from build123d import *

# Parameters (mm, degrees)
BASE_BLOCK_DEPTH             = 12
BASE_CHANNEL_CUT_30X15_DEPTH = 73
TAPERED_PEDESTAL_DEPTH       = 60
SADDLE_BODY_DEPTH            = 82
SADDLE_RECESS_CUT_DEPTH      = 20
SIDE_RELIEF_SKETCH_W         = 19.32494716
SIDE_RELIEF_SKETCH_H         = 14.354217055
SIDE_RELIEF_CUT_DEPTH        = 28


with BuildPart() as part:
    # Base Profile Sketch → Base Block (new body)
    with BuildSketch(Plane(origin=(0, 0, 0), x_dir=(1, 0, 0), z_dir=(0, 1, 0))):
        Polygon((0, 0), (30, 0), (30, 100), (-30, 100), (-30, 0), align=None)
    extrude(amount=BASE_BLOCK_DEPTH)

    # Base Channel Sketch → Base Channel Cut 30x15 (cut)
    with BuildSketch(Plane(origin=(0, 12, 0), x_dir=(1, 0, 0), z_dir=(0, 1, 0))):
        Polygon((0, 0), (15, 0), (15, 100), (-15, 100), (-15, 0), align=None)
    extrude(amount=-BASE_CHANNEL_CUT_30X15_DEPTH, mode=Mode.SUBTRACT)


with BuildPart() as base_channel_cut_30x15_piece_1:
    # of the separate pieces the step leaves, piece 1, a body of its own (base_channel_cut_30x15_pieces)
    add(part.part.solids().sort_by_distance((30, 0, 0))[0])



with BuildPart() as base_channel_cut_30x15_piece_2:
    # of the separate pieces the step leaves, piece 2, a body of its own (base_channel_cut_30x15_pieces)
    add(part.part.solids().sort_by_distance((-15, 12, 0))[0])


with BuildPart() as base_channel_cut_30x15_piece_1_1:
    add(base_channel_cut_30x15_piece_1.part)

    add(base_channel_cut_30x15_piece_2.part)  # Tapered Pedestal merges Base Channel Cut 30x15 piece 2
    # Pedestal Profile Sketch → Tapered Pedestal (add)
    with BuildSketch(Plane.XY.offset(-20)):
        with BuildLine():
            Line((0, 32), (25, 32))
            Line((25, 32), (30, 12))
            Line((30, 12), (15, 12))
            ThreePointArc((15, 12), (0, 27), (-15, 12))
            Line((-15, 12), (-30, 12))
            Line((-30, 12), (-25, 32))
            Line((-25, 32), (0, 32))
        make_face()
    extrude(amount=-TAPERED_PEDESTAL_DEPTH)

    # Saddle Profile Sketch → Saddle Body (add)
    with BuildSketch(Plane.XY.offset(-9)):
        with BuildLine():
            Line((10, 68), (20, 68))
            Line((20, 68), (25, 32))
            Line((25, 32), (-10.572876043, 32))
            Line((-10.572876043, 32), (-25, 32))
            Line((-25, 32), (-20, 68))
            Line((-20, 68), (-10, 68))
            ThreePointArc((-10, 68), (0, 58), (10, 68))
        make_face()
    extrude(amount=-SADDLE_BODY_DEPTH)

    # Saddle Recess Sketch → Saddle Recess Cut (cut)
    with BuildSketch(Plane(origin=(0, 68, 0), x_dir=(1, 0, 0), z_dir=(0, 1, 0))):
        Polygon((20, 75), (-20, 75), (-29.513236355, 75), (-29.513236355, 25), (-20, 25), (20, 25), (26.893267856, 25), (26.893267856, 75), align=None)
    extrude(amount=-SADDLE_RECESS_CUT_DEPTH, mode=Mode.SUBTRACT)

    # Side Relief Sketch → Side Relief Cut (cut)
    with BuildSketch(Plane(origin=(28.887206662, 4.012112036, 0), x_dir=(0, 0, -1), z_dir=(0.9904922731777517, 0.13756837127468668, 0))):
        with Locations((50, 28.25654346)):
            Rectangle(SIDE_RELIEF_SKETCH_W, SIDE_RELIEF_SKETCH_H)
    side_relief_cut = extrude(amount=-SIDE_RELIEF_CUT_DEPTH, mode=Mode.SUBTRACT)

    # Side Relief Mirror: Side Relief Cut across plane
    add(side_relief_cut.mirror(Plane(origin=(0, 0, 0), x_dir=(0, 0, 1), z_dir=(1, 0, 0))), mode=Mode.SUBTRACT)


solid = base_channel_cut_30x15_piece_1_1.part
Geometry check sheet. Reference: the model listing, model coordinates, mm. A direction names the side the tool comes from. Round coordinates to 2 decimals unless told otherwise and drop trailing zeros. Loops run counter-clockwise (first coordinate to the right, second up) from the corner with the lowest first, then second, coordinate; pieces in that order, holes last.
Item 1: Cross-section at A-A on z = -54.5. Record the boundary of the cut face in (x, y).
Item 2: Mould release check, pull along X, two halves, no side actions. Record for faces 4 (the flat face through (-23, 12, -90)), 5 (the flat face through (30, 6, -49)), 6 (the flat face through (18.34, 23.83, -49.86)): pulls with the +X half, pulls with the -X half, needs draft (parallel to the pull), parting line crosses it, or undercut.
Item 3: Gauge pin test, flat ends, axial feed: pin 1 (1 mm diameter, centred on x = 16, y = 42.5, fed in from -Z); pin 2 (18 mm diameter, centred on x = 4.5, y = 28.5, fed in from +Z); pin 3 (3.5 mm diameter, centred on x = 11.5, z = -86, fed in from -Y). Record the tip position at first contact, or that the pin passes through.
Item 4: Cross-section at D-D on y = 30.5. Record the boundary of the cut face in (x, z) (3 decimals), then the cut area to 3 significant figures.
Item 5: Access from +Z, -Z, +X, -X, +Y, -Y to the whole of each face (thin tool, end or side, straight path). Record for faces 1 (the flat face through (0, 29, -80)), 2 (the flat face through (-1, 32, -40.338)), 3 (the flat face through (0, 48, -50)).
Item 6: Cross-section at B-B on x = 17. Record the boundary of the cut face in (y, z), then the cut area to 3 significant figures.
Item 7: Cross-section at C-C on z = -86. Record the boundary of the cut face in (x, y), then the cut area to 3 significant figures.
Item 8: Thickness scan on line 1 (Y direction, x = 18, z = -90); line 2 (Z direction, x = -24, y = 28.5); line 3 (Z direction, x = 11, y = 62). Record the ranges inside material, lowest first.
Answer sheet:
1. outline: (-30, 0) - (-15, 0) - (-15, 12) arc R15 cw to (-10.47, 22.74) - (-25.99, 24.89) - (-25, 32) - (-30, 12) - close; (-24.01, 39.11) - (0, 35.77) - (24.01, 39.11) - (22.78, 48) - (-22.78, 48) - close; (10.47, 22.74) arc R15 cw to (15, 12) - (15, 0) - (30, 0) - (30, 12) - (25, 32) - (25.99, 24.89) - close
2. face 4: needs draft
2. face 5: pulls with the +X half
2. face 6: undercut
3. pin 1: stops at z = -91
3. pin 2: stops at z = -9
3. pin 3: stops at y = 32
4. outline: (-25.375, -80) - (25.375, -80) - (25.375, -20) - (-25.375, -20) - close; hole (-25.208, -59.662) - (25.208, -59.662) - (25.208, -40.338) - (-25.208, -40.338) - close
4. area: 2,070 mm2
5. face 1: -Z, +X, -X
5. face 2: none
5. face 3: +X, -X, +Y
6. outline: (0, -100) - (12, -100) - (12, -80) - (32, -80) - (32, -91) - (68, -91) - (68, -75) - (48, -75) - (48, -25) - (68, -25) - (68, -9) - (32, -9) - (32, -20) - (12, -20) - (12, 0) - (0, 0) - close; hole (23.64, -59.66) - (38.13, -59.66) - (38.13, -40.34) - (23.64, -40.34) - close
6. area: 4,070 mm2
7. outline: (-30, 0) - (-15, 0) - (-15, 12) - (-30, 12) - close; (-25, 32) - (25, 32) - (20, 68) - (10, 68) arc R10 cw to (-10, 68) - (-20, 68) - close; (15, 0) - (30, 0) - (30, 12) - (15, 12) - close
7. area: 1,820 mm2
8. line 1: y = 0 to 12, 32 to 68
8. line 2: z = -80 to -59.66, -40.34 to -20
8. line 3: z = -91 to -75, -25 to -9
